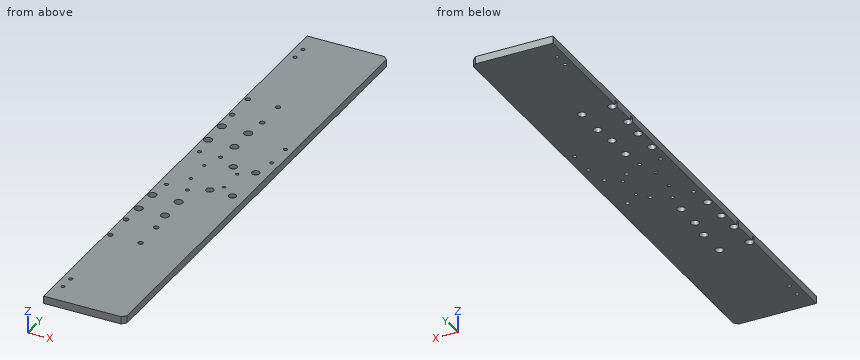
from build123d import *

# Parameters (mm, degrees)
SKETCH_1_W                     = 108
SKETCH_1_H                     = 675
EXTRUDE_1_DEPTH                = 10
HOLE_WIZARD_M6_1_D             = 5
HOLE_WIZARD_M6_1_2_D           = 6.6
HOLE_WIZARD_M6_1_2_CBORE_D     = 11
HOLE_WIZARD_M6_1_2_CBORE_DEPTH = 6.4
HOLE_WIZARD_M5_1_D             = 4.2
HOLE_WIZARD_M5_1_DEPTH         = 14
HOLE_WIZARD_M5_1_TIP           = 1.2618073
HOLE_WIZARD_M6_2_D             = 5
HOLE_WIZARD_M6_2_DEPTH         = 17
HOLE_WIZARD_M6_2_TIP           = 1.502151548
HOLE_WIZARD_M5_1_2_D           = 5.5
HOLE_WIZARD_M5_1_2_DEPTH       = 14
HOLE_WIZARD_M5_1_2_CBORE_D     = 10
HOLE_WIZARD_M5_1_2_CBORE_DEPTH = 5.4
HOLE_WIZARD_M5_1_2_TIP         = 1.652366702
HOLE_WIZARD_M6_3_D             = 5
HOLE_WIZARD_M6_3_DEPTH         = 17
HOLE_WIZARD_M6_3_TIP           = 1.502151548
SKETCH_14_R                    = 5.5
CUT_EXTRUDE_1_DEPTH            = 60
CHAMFER_1_SIZE                 = 5


with BuildPart() as part:
    # 草图1 → 凸台-拉伸1 (new body)
    with BuildSketch(Plane.XY):
        with Locations((54, 337.5)):
            Rectangle(SKETCH_1_W, SKETCH_1_H)
    extrude(amount=EXTRUDE_1_DEPTH)

    # Hole Wizard M6 _1 (through all)
    with Locations(Plane.XY.offset(10)):
        with Locations((10, 645), (10, 625), (10, 50), (10, 30)):
            Hole(HOLE_WIZARD_M6_1_D / 2)

    # Hole Wizard M6 _1 2 (through all)
    with Locations(Plane(origin=(0, 0, 0), x_dir=(-1, 0, 0), z_dir=(0, 0, -1))):
        with Locations((-45, 513.5), (-5, 513.5), (-45, 473.5), (-5, 473.5), (-5, 201.5), (-45, 201.5), (-5, 161.5), (-45, 161.5)):
            CounterBoreHole(HOLE_WIZARD_M6_1_2_D / 2, HOLE_WIZARD_M6_1_2_CBORE_D / 2, HOLE_WIZARD_M6_1_2_CBORE_DEPTH)

    # Hole Wizard M5 _1
    with Locations(Plane.XY.offset(10)):
        with Locations((29.5, 354.5), (73.5, 354.5), (29.5, 320.5), (73.5, 320.5)):
            Hole(HOLE_WIZARD_M5_1_D / 2, depth=HOLE_WIZARD_M5_1_DEPTH)
            with Locations((0, 0, -(HOLE_WIZARD_M5_1_DEPTH + HOLE_WIZARD_M5_1_TIP / 2))):  # 118° drill point
                Cone(0, HOLE_WIZARD_M5_1_D / 2, HOLE_WIZARD_M5_1_TIP, mode=Mode.SUBTRACT)

    # M6 螺纹孔2
    with Locations(Plane.XY.offset(10)):
        with Locations((97.5, 431.5), (97.5, 396.5)):
            Hole(HOLE_WIZARD_M6_2_D / 2, depth=HOLE_WIZARD_M6_2_DEPTH)
            with Locations((0, 0, -(HOLE_WIZARD_M6_2_DEPTH + HOLE_WIZARD_M6_2_TIP / 2))):  # 118° drill point
                Cone(0, HOLE_WIZARD_M6_2_D / 2, HOLE_WIZARD_M6_2_TIP, mode=Mode.SUBTRACT)

    # Hole Wizard M5 _1 2
    with Locations(Plane.XY.offset(10)):
        with Locations((61.5, 367.5), (91.5, 367.5), (61.5, 307.5), (91.5, 307.5)):
            CounterBoreHole(HOLE_WIZARD_M5_1_2_D / 2, HOLE_WIZARD_M5_1_2_CBORE_D / 2, HOLE_WIZARD_M5_1_2_CBORE_DEPTH, depth=HOLE_WIZARD_M5_1_2_DEPTH)
            with Locations((0, 0, -(HOLE_WIZARD_M5_1_2_DEPTH + HOLE_WIZARD_M5_1_2_TIP / 2))):  # 118° drill point
                Cone(0, HOLE_WIZARD_M5_1_2_D / 2, HOLE_WIZARD_M5_1_2_TIP, mode=Mode.SUBTRACT)

    # M6 螺纹孔3
    with Locations(Plane(origin=(0, 0, 0), x_dir=(-1, 0, 0), z_dir=(0, 0, -1))):
        with Locations((-38, 380), (-10, 380), (-38, 295), (-10, 295)):
            Hole(HOLE_WIZARD_M6_3_D / 2, depth=HOLE_WIZARD_M6_3_DEPTH)
            with Locations((0, 0, -(HOLE_WIZARD_M6_3_DEPTH + HOLE_WIZARD_M6_3_TIP / 2))):  # 118° drill point
                Cone(0, HOLE_WIZARD_M6_3_D / 2, HOLE_WIZARD_M6_3_TIP, mode=Mode.SUBTRACT)

    # 草图14 → 切除-拉伸1 (cut)
    with BuildSketch(Plane.XY.offset(10)):
        with Locations((41.5, 444)):
            Circle(SKETCH_14_R)
        with Locations((6.5, 444)):
            Circle(SKETCH_14_R)
        with Locations((41.5, 409)):
            Circle(SKETCH_14_R)
        with Locations((6.5, 409)):
            Circle(SKETCH_14_R)
        with Locations((41.5, 266)):
            Circle(SKETCH_14_R)
        with Locations((41.5, 231)):
            Circle(SKETCH_14_R)
        with Locations((6.5, 231)):
            Circle(SKETCH_14_R)
        with Locations((6.5, 266)):
            Circle(SKETCH_14_R)
    extrude(amount=-CUT_EXTRUDE_1_DEPTH, mode=Mode.SUBTRACT)

    # 倒角1
    chamfer_1_edges = [part.edges().sort_by_distance(p)[0] for p in [
        (108, 0, 5),
        (108, 675, 5),
    ]]
    chamfer(chamfer_1_edges, length=CHAMFER_1_SIZE)


solid = part.part
Here's how the part is built. I have some questions about the finished solid (model axes, mm). Round coordinates to 2 decimals unless told otherwise and drop trailing zeros. Return JSON: item names as keys, results as strings.
Q1. If we section it at A-A on z = 2.25: Give the number of separate pieces and of enclosed holes in the cut face, plus the area to 3 significant figures.
Filled sheet:
{"separate pieces": "1", "enclosed holes": "30", "area": "71,000 mm^2"}
Q2. For pin 1 Ø3 at (x, y) = (6, 516) entering from -Z; pin 2 Ø4 at (x, y) = (45, 201.5) entering from +Z; pin 3 Ø9 at (x, y) = (91.5, 367.5) entering from +Z, each with a flat end and sliding along its axis, tell me the tip position at first contact or that it passes through.
Filled sheet:
{"pin 1": "stops at z = 6.4", "pin 2": "passes through", "pin 3": "stops at z = 4.6"}
Q3. I need wall thicknesses on line 1 along Y through (x, z) = (91.5, 2.6); line 2 along X through (y, z) = (295, 2.25); line 3 along X through (y, z) = (410, 4.5). Which ranges of each line are inside material? Lowest first, please. Write a range as from..to.
Filled sheet:
{"line 1": "y = 0..304.75, 310.25..364.75, 370.25..675", "line 2": "x = 0..7.5, 12.5..35.5, 40.5..108", "line 3": "x = 0..1.09, 11.91..36.09, 46.91..108"}
